Check sheet for the modelled part. Datum: model origin and axes. Units: mm. Face numbers are marked on the shaded views. A direction names the side the tool comes from. Round coordinates to 2 decimals unless told otherwise and drop trailing zeros. Loops run counter-clockwise (first coordinate to the right, second up) from the corner with the lowest first, then second, coordinate; pieces in that order, holes last. Notation, with made-up numbers: (35.25, -14) - (58.25, -14) arc R19 cw to (58.25, 18) - close; hole circle Ø2 at (-29, -16). An arc over 180 degrees is marked (long way). Put each result on its own line as item: value.
```python
from build123d import *

# Parameters (mm, degrees)
BACK_PLATE_SKETCH_W      = 20
BACK_PLATE_SKETCH_H      = 16
BACK_PLATE_16X20X2_DEPTH = 2
BRACKET_PROFILE_SKETCH_R = 1
HOOK_BRACKET_DEPTH       = 2
PIN_CIRCLES_SKETCH_R     = 1
MOUNTING_PINS_2X_DEPTH   = 5
HOOK_SECTION_SKETCH_W    = 2
HOOK_SECTION_SKETCH_H    = 2
HOOK_TIP_DEPTH           = 2


with BuildPart() as part:
    # Back Plate Sketch → Back Plate 16x20x2 (new body)
    with BuildSketch(Plane.XY):
        Rectangle(BACK_PLATE_SKETCH_W, BACK_PLATE_SKETCH_H)
    extrude(amount=BACK_PLATE_16X20X2_DEPTH)

    # Bracket Profile Sketch → Hook Bracket (add)
    with BuildSketch(Plane.XY.offset(2)):
        with BuildLine():
            Line((-1, -3), (-1, -8))
            Line((-1, -8), (1, -8))
            Line((1, -8), (1, -3))
            ThreePointArc((1, -3), (3.84680434, -1.051653316), (7.06343132, 0.19480592))
            ThreePointArc((7.06343132, 0.19480592), (8.770582601, 4.150596389), (4.76336302, 5.73326343))
            ThreePointArc((4.76336302, 5.73326343), (0, 5.15774213), (-4.76336302, 5.73326343))
            ThreePointArc((-4.76336302, 5.73326343), (-8.770582601, 4.150596389), (-7.06343132, 0.19480592))
            ThreePointArc((-7.06343132, 0.19480592), (-3.84680434, -1.051653316), (-1, -3))
        make_face()
        with Locations((-6, 3)):
            Circle(BRACKET_PROFILE_SKETCH_R, mode=Mode.SUBTRACT)
        with Locations(Location((6, 3, 0), (0, 0, 180))):
            Circle(BRACKET_PROFILE_SKETCH_R, mode=Mode.SUBTRACT)
    extrude(amount=HOOK_BRACKET_DEPTH)

    # Pin Circles Sketch → Mounting Pins 2x (add)
    with BuildSketch(Plane.XY.offset(2)):
        with Locations((-6, 3)):
            Circle(PIN_CIRCLES_SKETCH_R)
        with Locations(Location((6, 3, 0), (0, 0, 180))):
            Circle(PIN_CIRCLES_SKETCH_R)
    extrude(amount=MOUNTING_PINS_2X_DEPTH)

    # Hook Arm Sweep: sweep along a path in Hook Path Sketch
    with BuildLine(Plane(origin=(0, 0, 0), x_dir=(0, 0, -1), z_dir=(1, 0, 0))) as hook_arm_sweep_path:
        ThreePointArc((-3, -8), (-12, -17), (-21, -8))
    # Hook Section Sketch → Hook Arm Sweep (sweep)
    with BuildSketch(Plane.XZ.offset(8)):
        with Locations((0, 3)):
            Rectangle(HOOK_SECTION_SKETCH_W, HOOK_SECTION_SKETCH_H)
    sweep(path=hook_arm_sweep_path.line)

    # Hook Tip Sketch → Hook Tip (add)
    with BuildSketch(Plane.ZY.offset(1)):
        with BuildLine():
            Line((20, -8), (22, -8))
            ThreePointArc((22, -8), (21, -7), (20, -8))
        make_face()
    extrude(amount=-HOOK_TIP_DEPTH)


solid = part.part
```
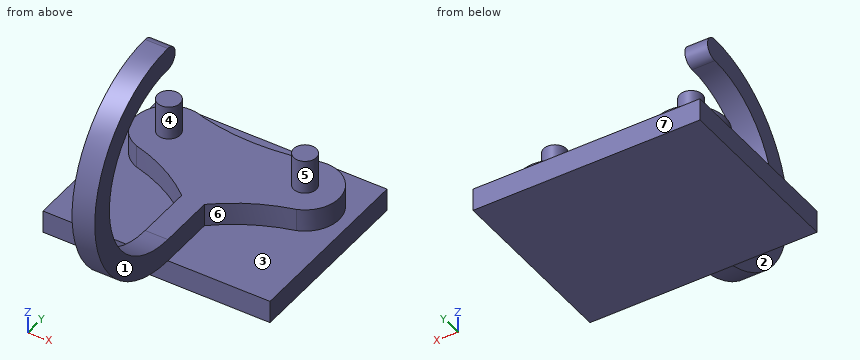
Item 1: Section check D-D on z = 4.5. Enter the section's corners in (x, y), then the cut area to 3 significant figures.
Filled sheet:
outline: circle Ø2 at (-6, 3); (-1, -14.61) - (1, -14.61) - (1, -10.78) - (-1, -10.78) - close; circle Ø2 at (6, 3)
area: 13.9 mm²
Item 2: Tool access check on the marked faces 1, 2 and 3. Record the directions out of +Z, -Z, +X, -X, +Y, -Y that give a thin tool (end or side, any length) a straight path to the whole face; none if there is none.
Filled sheet:
face 1: +Z, +X, -Y
face 2: +Z, -X, -Y
face 3: +Z
Item 3: Go/stop test with flat-tipped pins: pin 1 (2 mm diameter, centred on x = 3, z = 1.5, fed in from -Y); pin 2 (6 mm diameter, centred on x = -2, z = 10, fed in from +Y); pin 3 (0.6 mm diameter, centred on x = 5.5, y = 3.5, fed in from +Z). Record where each tip stops, or that it passes through.
Filled sheet:
pin 1: y = -8
pin 2: y = -14.38
pin 3: z = 7
Item 4: Section check C-C on x = 6. Enter the section's corners in (y, z), then the cut area to 3 significant figures.
Filled sheet:
outline: (-8, 0) - (8, 0) - (8, 2) - (6, 2) - (6, 4) - (4, 4) - (4, 7) - (2, 7) - (2, 4) - (-0.12, 4) - (-0.12, 2) - (-8, 2) - close
area: 50.2 mm²
Item 5: Release check for a two-part mould opening along X. For the marked faces 4, 5, 6 and 7 record: +X half, -X half, draft (parallel to the pull), parting line (faces both ways), or undercut.
Filled sheet:
face 4: undercut
face 5: undercut
face 6: +X half
face 7: draft
Item 6: Section check B-B on y = 3. Enter the section's corners in (x, z).
Filled sheet:
outline: (-10, 0) - (10, 0) - (10, 2) - (9, 2) - (9, 4) - (7, 4) - (7, 7) - (5, 7) - (5, 4) - (-5, 4) - (-5, 7) - (-7, 7) - (-7, 4) - (-9, 4) - (-9, 2) - (-10, 2) - close
Item 7: Thickness scan on line 1 (X direction, y = -11.75, z = 3.75); line 2 (Z direction, x = -3, y = -2); line 3 (Z direction, x = -2, y = -1). Record the ranges inside material, lowest first. Write a range as from..to.
Filled sheet:
line 1: -1..1
line 2: 0..2
line 3: 0..4
Item 8: Section check A-A on y = -15.5. Enter the section's corners in (x, z).
Filled sheet:
outline: (-1, 5.39) - (1, 5.39) - (1, 9.22) - (-1, 9.22) - close; (-1, 14.78) - (1, 14.78) - (1, 18.61) - (-1, 18.61) - close
